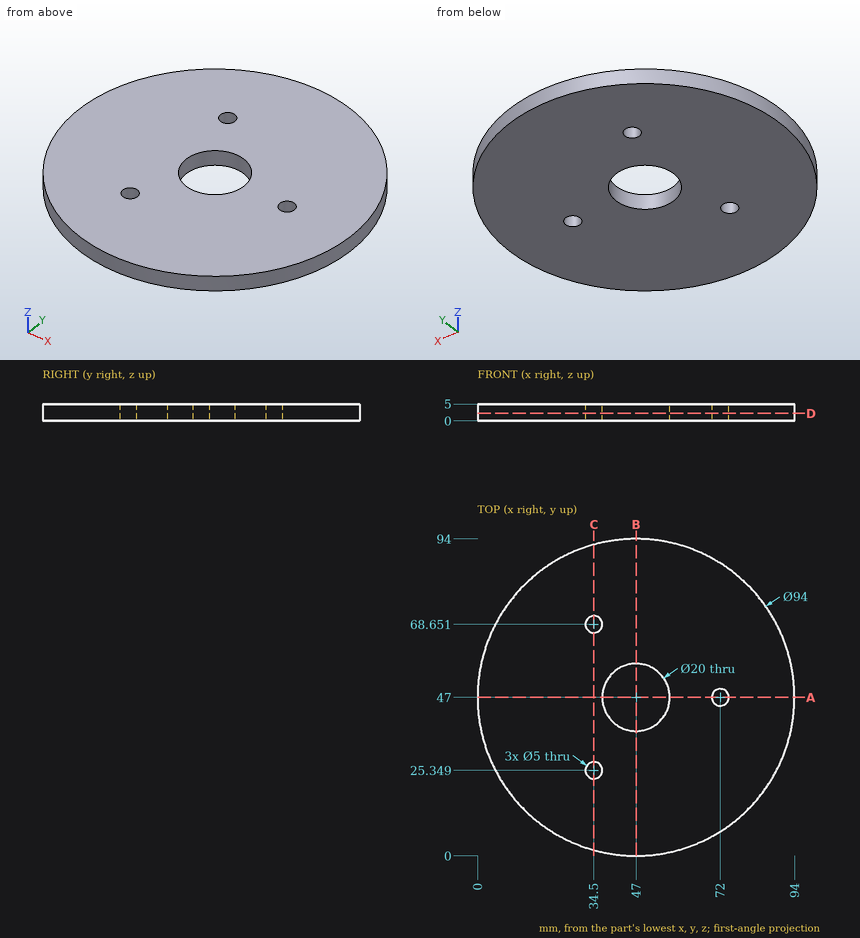
Geometry check sheet. Reference: drawing and pictorial views, mm from the part's lowest x, y, z. Coordinates: 2 decimals unless noted, no trailing zeros. Order: outer loops, then holes, each group sorted by start corner. A loop starts at its lowest first (then second) coordinate and runs counter-clockwise, first axis right, second up. Notation, with made-up numbers: (-33.5, -33) -> (-28.5, -33) arc R15 ccw to (-28.5, -6) -> close; hole circle Ø8 at (61.25, 64.25). An arc over 180 degrees is marked (long way). Write item = value, one per line. Start each with the question number.
1) Cross-section at D-D (z = 2.2). Enter the section's corners in (x, y).
2) Go/stop test with a flat-tipped pin: P1, Ø1, axis at y = 44, z = 2.5, coming from the +X side. Record where the tip stops, or that it passes through.
3) Cross-section at C-C (x = 34.5). Enter the section's corners in (y, z).
4) Cross-section at A-A (y = 47). Enter the section's corners in (x, z).
5) Material ranges on L1, parallel to Y at x = 34.5, z = 1.15; L2, parallel to X at y = 47.5, z = 1.1; L3, parallel to Y at x = 47, z = 3.6, recorded low to high.
6) Cross-section at B-B (x = 47). Enter the section's corners in (y, z), then the cut area to 3 significant figures.
Ans:
q1.outline = circle Ø94 at (47, 47); hole circle Ø5 at (34.5, 25.35); hole circle Ø5 at (34.5, 68.65); hole circle Ø20 at (47, 47); hole circle Ø5 at (72, 47)
q2.P1 = 93.93
q3.outline = (1.69, 0) -> (22.85, 0) -> (22.85, 5) -> (1.69, 5) -> close; (27.85, 0) -> (66.15, 0) -> (66.15, 5) -> (27.85, 5) -> close; (71.15, 0) -> (92.31, 0) -> (92.31, 5) -> (71.15, 5) -> close
q4.outline = (0, 0) -> (37, 0) -> (37, 5) -> (0, 5) -> close; (57, 0) -> (69.5, 0) -> (69.5, 5) -> (57, 5) -> close; (74.5, 0) -> (94, 0) -> (94, 5) -> (74.5, 5) -> close
q5.L1 = 1.69 to 22.85, 27.85 to 66.15, 71.15 to 92.31
q5.L2 = 0 to 37.01, 56.99 to 69.55, 74.45 to 94
q5.L3 = 0 to 37, 57 to 94
q6.outline = (0, 0) -> (37, 0) -> (37, 5) -> (0, 5) -> close; (57, 0) -> (94, 0) -> (94, 5) -> (57, 5) -> close
q6.area = 370 mm²
